Design review of the part built by this model. Coordinates are the model's own, in mm. Face numbers are marked on the shaded views. A direction names the side the tool comes from. Round coordinates to 2 decimals unless told otherwise and drop trailing zeros. Order: outer loops, then holes, each group sorted by start corner. A loop starts at its lowest first (then second) coordinate and runs counter-clockwise, first axis right, second up. Notation, with made-up numbers: (8, 26) - (62, 26) arc R23 cw to (62, 47) - close; hole circle Ø3 at (73, 41). An arc over 180 degrees is marked (long way). Write item = value, one per line.
from build123d import *

# Parameters (mm, degrees)
EXTRUDE_1_DEPTH           = 18
SKETCH_2_W                = 38
SKETCH_2_H                = 32
CUT_EXTRUDE_1_DEPTH       = 1.5
HOLE_WIZARD_1_D           = 4.5
HOLE_WIZARD_1_CBORE_D     = 8
HOLE_WIZARD_1_CBORE_DEPTH = 4.6


with BuildPart() as part:
    # 草图1 → 凸台-拉伸1 (new, symmetric)
    with BuildSketch(Plane.XY):
        Polygon((0, 0), (-19, 0), (-19, 10), (-5, 10), (-5, 50), (5, 50), (5, 10), (19, 10), (19, 0), align=None)
    extrude(amount=EXTRUDE_1_DEPTH, both=True)

    # 草图2 → 切除-拉伸1 (cut)
    with BuildSketch(Plane.XZ):
        Rectangle(SKETCH_2_W, SKETCH_2_H)
    extrude(amount=-CUT_EXTRUDE_1_DEPTH, mode=Mode.SUBTRACT)

    # 打孔尺寸(%根据)内六角圆柱头螺钉的类型1 (through all)
    with Locations(Plane(origin=(-10, 10, 12), x_dir=(0, 0, 1), z_dir=(0, 1, 0))):
        with Locations((0, 0)):
            CounterBoreHole(HOLE_WIZARD_1_D / 2, HOLE_WIZARD_1_CBORE_D / 2, HOLE_WIZARD_1_CBORE_DEPTH)


solid = part.part
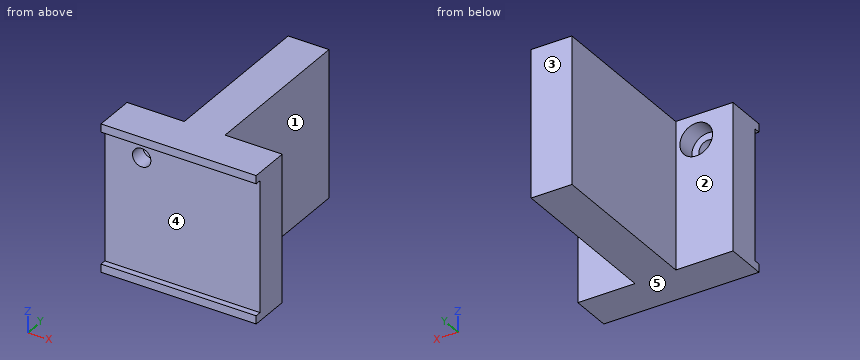
Item 1: For the marked faces 1, 2, 3, 4 and 5, list the 3-axis set-ups (+Z, -Z, +X, -X, +Y, -Y) from which the entire face can be reached by the end or side of a thin tool; tool diameter is ignored.
Data:
face_1 = +Z, -Z, +X, +Y
face_2 = +Z, -Z, -X, +Y
face_3 = +Z, -Z, +X, -X, +Y
face_4 = +X, -X, -Y
face_5 = -Z, +X, -X, +Y, -Y
Item 2: For line 1 along X through (y, z) = (4, 12); line 2 along X through (y, z) = (8.75, 12); line 3 along Y through (x, z) = (10, 4), list the stretches that pass through material, from the lowest coordinate up. Write a range as [from, to].
Data:
line_1 = [-19, -12.25], [-7.75, 19]
line_2 = [-19, -14], [-6, 19]
line_3 = [1.5, 10]
Item 3: Take a section at D-D, the plane x = 14. State the section outline as (y, z) points, and give its area (3 significant figures).
Data:
outline = (0, -18) - (10, -18) - (10, 18) - (0, 18) - (0, 16) - (1.5, 16) - (1.5, -16) - (0, -16) - close
area = 312 mm2
Item 4: Take a section at A-A, the plane z = 12. State the section outline as (x, y) points, and give its area (3 significant figures).
Data:
outline = (-19, 1.5) - (-12.25, 1.5) - (-12.25, 5.4) - (-14, 5.4) - (-14, 10) - (-19, 10) - close; (-7.75, 1.5) - (19, 1.5) - (19, 10) - (5, 10) - (5, 50) - (-5, 50) - (-5, 10) - (-6, 10) - (-6, 5.4) - (-7.75, 5.4) - close
area = 669 mm2
Item 5: Take a section at B-B, the plane x = -10. State the section outline as (y, z) points.
Data:
outline = (0, -18) - (10, -18) - (10, 8) - (5.4, 8) - (5.4, 9.75) - (1.5, 9.75) - (1.5, -16) - (0, -16) - close; (0, 16) - (1.5, 16) - (1.5, 14.25) - (5.4, 14.25) - (5.4, 16) - (10, 16) - (10, 18) - (0, 18) - close
Item 6: Take a section at C-C, the plane z = -7. State the section outline as (x, y) points.
Data:
outline = (-19, 1.5) - (19, 1.5) - (19, 10) - (5, 10) - (5, 50) - (-5, 50) - (-5, 10) - (-19, 10) - close
Item 7: Insertion check: P1, Ø9.5, axis at x = 1, z = -7, coming from the -Y side; P2, Ø2, axis at y = 37.5, z = 11.5, coming from the +X side; P3, Ø5, axis at x = -10, z = 12, coming from the +Y side. Each pin has a flat end and moves straight along its axis. Give the tip position at first contact, or say it passes through.
Data:
P1 = 1.5
P2 = 5
P3 = 5.4
